Can you work these out from the drawing? Everything is in mm from the part's minimum corner. A direction names the side the tool comes from. Round coordinates to 2 decimals unless told otherwise and drop trailing zeros. Order: outer loops, then holes, each group sorted by start corner. A loop starts at its lowest first (then second) coordinate and runs counter-clockwise, first axis right, second up. Notation, with made-up numbers: (-35.5, 16.25) - (-18.5, 16.25) arc R29 ccw to (-18.5, 42.25) - close; hole circle Ø5 at (-39, 62.25). An arc over 180 degrees is marked (long way). Answer as a JSON object with one key per item and string values.
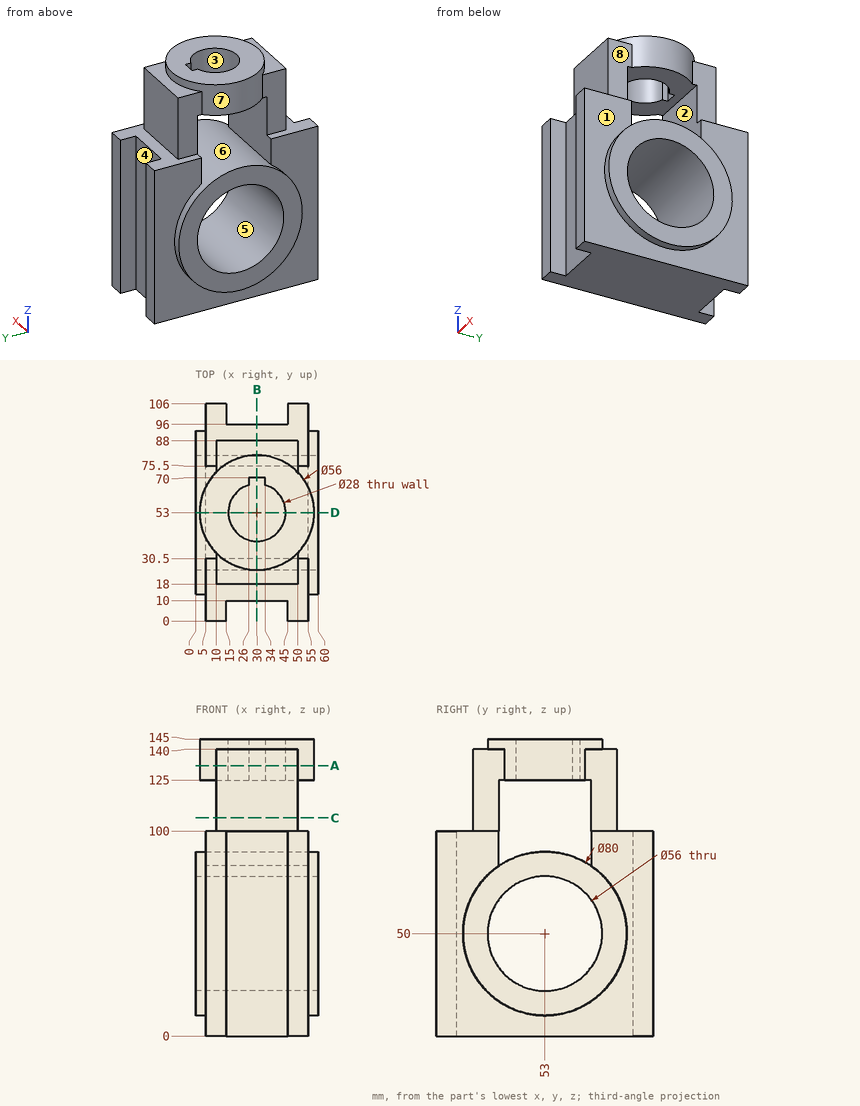
1. Imagine slicing it at A-A (z = 132). List the corners of the cut face in (x, y) for me, plus the area to 3 significant figures.
Responses:
{"outline": "(10, 18) - (50, 18) - (50, 33.4) arc R28 ccw to (50, 72.6) - (50, 88) - (10, 88) - (10, 72.6) arc R28 ccw to (10, 33.4) - close; hole (26, 66.42) arc R14 ccw (long way) to (34, 66.42) - (34, 70) - (26, 70) - close", "area": "2,590 mm2"}
2. For P1, Ø3, axis at y = 99, z = 58, coming from the +X side; P2, Ø4, axis at x = 10, y = 23.5, coming from the +Z side; P3, Ø6, axis at y = 25.5, z = 121.5, coming from the -X side; P4, Ø24, axis at x = 36.5, z = 63.5, coming from the -Y side, each with a flat end and sliding along its axis, tell me the tip position at first contact or that it passes through.
Responses:
{"P1": "x = 55", "P2": "z = 140", "P3": "x = 10", "P4": "y = 0"}
3. Imagine slicing it at C-C (z = 106.5). List the corners of the cut face in (x, y) for me, plus the area to 3 significant figures.
Responses:
{"outline": "(10, 18) - (50, 18) - (50, 30.5) - (10, 30.5) - close; (10, 75.5) - (50, 75.5) - (50, 88) - (10, 88) - close", "area": "1,000 mm2"}
4. For the marked faces 1, 2, 3 and 4, which set-ups out of +Z, -Z, +X, -X, +Y, -Y let a thin tool reach every point of the face, with its end or its side?
Responses:
{"face 1": "+X", "face 2": "+X, -X", "face 3": "+Z", "face 4": "+Z, -Z, +Y"}
5. Imagine slicing it at B-B (x = 30). List the corners of the cut face in (y, z) for me, plus the area to 3 significant figures.
Responses:
{"outline": "(10, 0) - (96, 0) - (96, 100) - (88, 100) - (88, 140) - (81, 140) - (81, 145) - (70, 145) - (70, 125) - (75.5, 125) - (75.5, 83.07) arc R40 ccw to (30.5, 83.07) - (30.5, 125) - (39, 125) - (39, 145) - (25, 145) - (25, 140) - (18, 140) - (18, 100) - (10, 100) - close; hole circle Ø56 at (53, 50)", "area": "6,920 mm2"}
6. If I drill on L1, parallel to Y at x = 30, z = 130.5; L2, parallel to Z at x = 50.5, y = 34; L3, parallel to X at y = 5.5, z = 88.5, over which ranges is the centre line in solid material (lowest first)? Write a range as [from, to].
Responses:
{"L1": "[18, 39], [70, 88]", "L2": "[0, 29.43], [70.57, 85.2], [125, 145]", "L3": "[5, 15], [45, 55]"}
7. Imagine slicing it at D-D (y = 53). List the corners of the cut face in (x, z) for me, plus the area to 3 significant figures.
Responses:
{"outline": "(0, 10) - (5, 10) - (5, 0) - (55, 0) - (55, 10) - (60, 10) - (60, 22) - (0, 22) - close; (0, 78) - (60, 78) - (60, 90) - (0, 90) - close; (2, 125) - (16, 125) - (16, 145) - (2, 145) - close; (44, 125) - (58, 125) - (58, 145) - (44, 145) - close", "area": "2,500 mm2"}
8. Thinking about a two-plate mould opening in Y: for the marked faces 5, 6, 7 and 8, which applies, pulls with the +Y half, pulls with the -Y half, needs draft (parallel to the pull), parting line crosses it, or undercut?
Responses:
{"face 5": "undercut", "face 6": "undercut", "face 7": "parting line crosses it", "face 8": "needs draft"}
